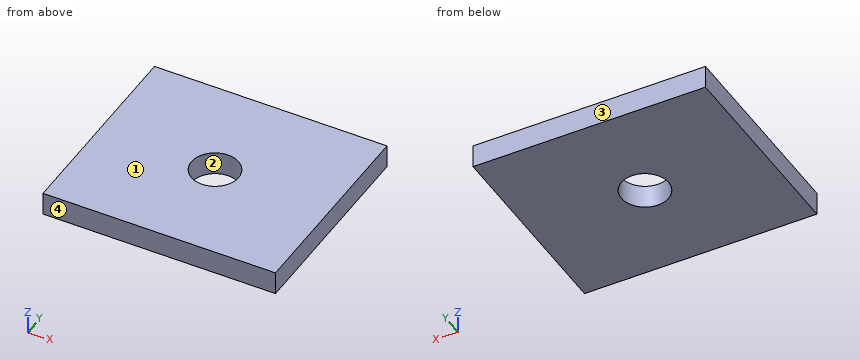
from build123d import *

# Parameters (mm, degrees)
SKETCH_1_W          = 80
SKETCH_1_H          = 70
EXTRUDE_1_DEPTH     = 4
SKETCH_2_R          = 8.1
CUT_EXTRUDE_1_DEPTH = 14


with BuildPart() as part:
    # 草图1 → 凸台-拉伸1 (new, symmetric)
    with BuildSketch(Plane.XY):
        Rectangle(SKETCH_1_W, SKETCH_1_H)
    extrude(amount=EXTRUDE_1_DEPTH, both=True)

    # 草图2 → 切除-拉伸1 (cut, symmetric)
    with BuildSketch(Plane.XY):
        Circle(SKETCH_2_R)
    extrude(amount=CUT_EXTRUDE_1_DEPTH, both=True, mode=Mode.SUBTRACT)


solid = part.part
Verification items for the finished model (mm, model axes). Face numbers are marked on the shaded views. Give positions to 0.01 mm unless a question says otherwise; leave off trailing zeros. Loops run counter-clockwise (first coordinate to the right, second up) from the corner with the lowest first, then second, coordinate; pieces in that order, holes last.
1. Cross-section at B-B on z = 0.5. Record the cut outline in (x, y).
Derived:
outline: (-40, -35) - (40, -35) - (40, 35) - (-40, 35) - close; hole circle Ø16.2 at (0, 0)
2. Go/stop test with a flat-tipped pin: P1, Ø9.5, axis at x = 0, y = 0, coming from the +Z side. Record where the tip stops, or that it passes through.
Derived:
P1: passes through
3. Cross-section at A-A on y = 0. Record the cut outline in (x, z).
Derived:
outline: (-40, -4) - (-8.1, -4) - (-8.1, 4) - (-40, 4) - close; (8.1, -4) - (40, -4) - (40, 4) - (8.1, 4) - close
4. Material ranges on probe 1 along Y at (x, z) = (0, 2); probe 2 along X at (y, z) = (-1, 2.75); probe 3 along Y at (x, z) = (-5.5, 2.75), recorded low to high.
Derived:
probe 1: y = -35 to -8.1, 8.1 to 35
probe 2: x = -40 to -8.04, 8.04 to 40
probe 3: y = -35 to -5.95, 5.95 to 35
5. Cross-section at C-C on x = 0. Record the cut outline in (y, z).
Derived:
outline: (-35, -4) - (-8.1, -4) - (-8.1, 4) - (-35, 4) - close; (8.1, -4) - (35, -4) - (35, 4) - (8.1, 4) - close
6. Release check for a two-part mould opening along Y. For the marked faces 1, 2, 3 and 4 record: +Y half, -Y half, draft (parallel to the pull), parting line (faces both ways), or undercut.
Derived:
face 1: draft
face 2: undercut
face 3: +Y half
face 4: -Y half
